Could you check a few things on this drawing? It's one solid part, dimensions in mm from its lowest x, y, z. A direction names the side the tool comes from. Give positions to 0.01 mm unless a question says otherwise; leave off trailing zeros. Order: outer loops, then holes, each group sorted by start corner. A loop starts at its lowest first (then second) coordinate and runs counter-clockwise, first axis right, second up. Notation, with made-up numbers: (68, 35) -> (118, 35) arc R14 cw to (118, 48) -> close; hole circle Ø6 at (79.25, 65.5). An arc over 180 degrees is marked (long way). Use one line per item in the form item = value. Start each with the question number.
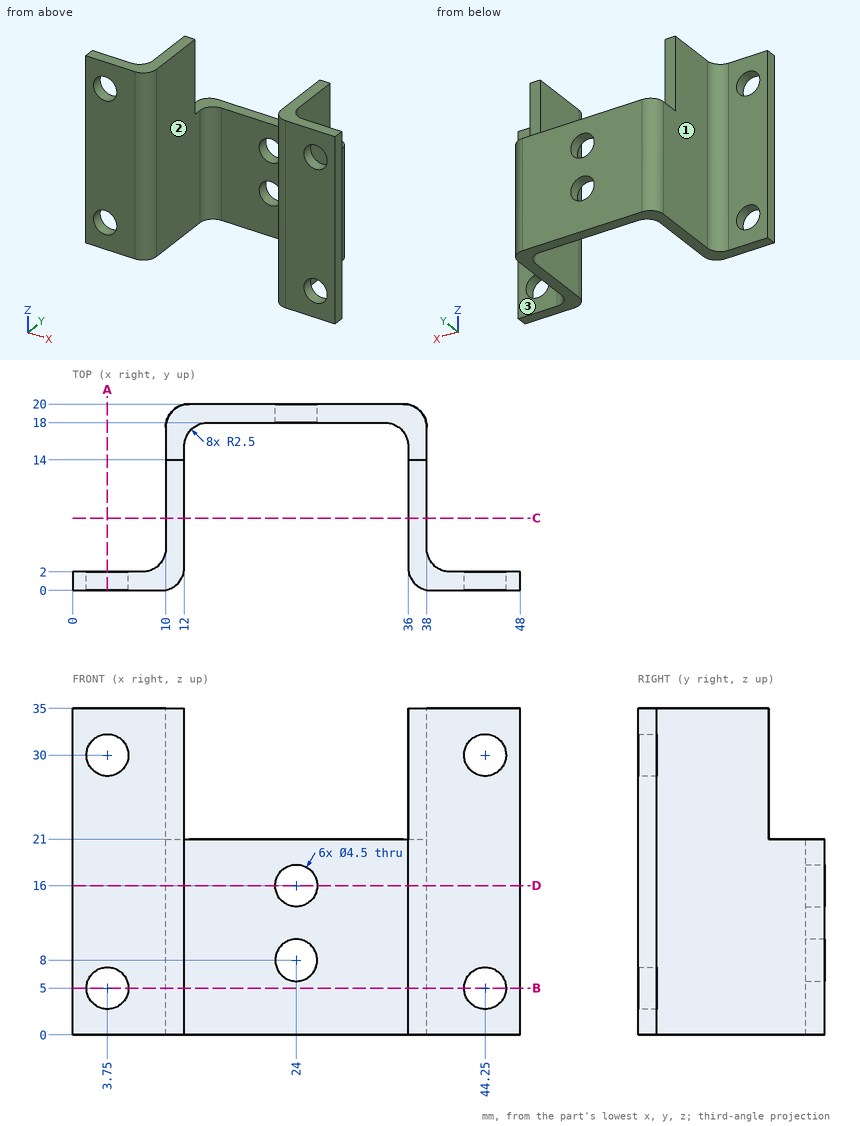
(1) Imagine slicing it at D-D (z = 16). Write out the boundary of the cut face in (x, y).
(2) Imagine slicing it at C-C (y = 7.75). Write out the boundary of the cut face in (x, z).
(3) I'm going to push flat-ended pins straight in: pin 1 Ø4 at (y, z) = (14, 6.5) entering from -X; pin 2 Ø8 at (x, z) = (25, 20.5) entering from -Y; pin 3 Ø4 at (x, z) = (24, 16) entering from -Y; pin 4 Ø8 at (x, z) = (43.5, 19) entering from +Y. Where does each tip first touch, or does it pass through?
(4) Which directions (+Z, -Z, +X, -X, +Y, -Y) give clear straight access to the entire face, cutting with the end or side of a thin tool? Please do the marked faces 1, 2 and 3.
(5) Imagine slicing it at B-B (z = 5). Write out the boundary of the cut face in (x, y).
(6) Imagine slicing it at A-A (x = 3.75). Write out the boundary of the cut face in (y, z), plus the area to 3 significant figures.
(7) Please list where these lines run through material, in increasing order: probe 1 along Z at (x, y) = (3.75, 1.45); probe 2 along X at (y, z) = (15, 2.5); probe 3 along X at (y, z) = (1.5, 5).
Calculated:
q1.outline = (0, 0) -> (9.5, 0) arc R2.5 ccw to (12, 2.5) -> (12, 15.5) arc R2.5 cw to (14.5, 18) -> (21.75, 18) -> (21.75, 20) -> (12.5, 20) arc R2.5 ccw to (10, 17.5) -> (10, 4.5) arc R2.5 cw to (7.5, 2) -> (0, 2) -> close; (26.25, 18) -> (33.5, 18) arc R2.5 cw to (36, 15.5) -> (36, 2.5) arc R2.5 ccw to (38.5, 0) -> (48, 0) -> (48, 2) -> (40.5, 2) arc R2.5 cw to (38, 4.5) -> (38, 17.5) arc R2.5 ccw to (35.5, 20) -> (26.25, 20) -> close
q2.outline = (10, 0) -> (12, 0) -> (12, 35) -> (10, 35) -> close; (36, 0) -> (38, 0) -> (38, 35) -> (36, 35) -> close
q3.pin_1 = 10
q3.pin_2 = 18
q3.pin_3 = through
q3.pin_4 = 2.21
q4.face_1 = +Z, -Z, -X, +Y
q4.face_2 = +Z, -Z, -Y
q4.face_3 = +Z, -Z, +X, +Y
q5.outline = (0, 0) -> (1.5, 0) -> (1.5, 2) -> (0, 2) -> close; (6, 0) -> (9.5, 0) arc R2.5 ccw to (12, 2.5) -> (12, 15.5) arc R2.5 cw to (14.5, 18) -> (33.5, 18) arc R2.5 cw to (36, 15.5) -> (36, 2.5) arc R2.5 ccw to (38.5, 0) -> (42, 0) -> (42, 2) -> (40.5, 2) arc R2.5 cw to (38, 4.5) -> (38, 17.5) arc R2.5 ccw to (35.5, 20) -> (12.5, 20) arc R2.5 ccw to (10, 17.5) -> (10, 4.5) arc R2.5 cw to (7.5, 2) -> (6, 2) -> close; (46.5, 0) -> (48, 0) -> (48, 2) -> (46.5, 2) -> close
q6.outline = (0, 0) -> (2, 0) -> (2, 2.75) -> (0, 2.75) -> close; (0, 7.25) -> (2, 7.25) -> (2, 27.75) -> (0, 27.75) -> close; (0, 32.25) -> (2, 32.25) -> (2, 35) -> (0, 35) -> close
q6.area = 52.0 mm2
q7.probe_1 = 0 to 2.75, 7.25 to 27.75, 32.25 to 35
q7.probe_2 = 10 to 12, 36 to 38
q7.probe_3 = 0 to 1.5, 6 to 11.79, 36.21 to 42, 46.5 to 48
